from build123d import *

# Parameters (mm, degrees)
SKETCH_1_W             = 500
SKETCH_1_H             = 300
EXTRUDE_1_DEPTH        = 45
SKETCH_2_R             = 22.5
CUT_EXTRUDE_1_DEPTH    = 8
CHAMFER_1_SIZE         = 3
SKETCH_16_R            = 15.5
CUT_EXTRUDE_3_DEPTH    = 296
SKETCH_17_R            = 31
CUT_EXTRUDE_4_DEPTH    = 296
HOLE_WIZARD_M4_1_D     = 3.3
HOLE_WIZARD_M4_1_DEPTH = 11
HOLE_WIZARD_M4_1_TIP   = 0.991420021
HOLE_WIZARD_M5_1_D     = 4.2
HOLE_WIZARD_M5_1_DEPTH = 13
HOLE_WIZARD_M5_1_TIP   = 1.2618073
HOLE_WIZARD_M30_1_D    = 26.5


with BuildPart() as part:
    # 草图1 → 凸台-拉伸1 (new body)
    with BuildSketch(Plane(origin=(0, 0, 0), x_dir=(1, 0, 0), z_dir=(0, 1, 0))):
        Rectangle(SKETCH_1_W, SKETCH_1_H)
    extrude(amount=EXTRUDE_1_DEPTH)

    # 草图2 → 切除-拉伸1 (cut)
    with BuildSketch(Plane.XZ):
        with Locations(Location((190, 90, 0), (0, 0, 270))):
            Circle(SKETCH_2_R)
        with Locations(Location((-190, 90, 0), (0, 0, 90))):
            Circle(SKETCH_2_R)
        with Locations(Location((190, -90, 0), (0, 0, 270))):
            Circle(SKETCH_2_R)
        with Locations(Location((-190, -90, 0), (0, 0, 90))):
            Circle(SKETCH_2_R)
    extrude(amount=-CUT_EXTRUDE_1_DEPTH, mode=Mode.SUBTRACT)

    # 倒角1
    chamfer_1_edges = [part.edges().sort_by_distance(p)[0] for p in [
        (250, 22.5, 150),
        (-250, 22.5, 150),
        (-250, 22.5, -150),
        (250, 22.5, -150),
    ]]
    chamfer(chamfer_1_edges, length=CHAMFER_1_SIZE)

    # 草图16 → 切除-拉伸3 (cut, through all)
    with BuildSketch(Plane(origin=(0, 45, 0), x_dir=(1, 0, 0), z_dir=(0, 1, 0))):
        with Locations(Location((190, -90, 0), (0, 0, 270))):
            Circle(SKETCH_16_R)
        with Locations(Location((190, 90, 0), (0, 0, 270))):
            Circle(SKETCH_16_R)
        with Locations(Location((-190, 90, 0), (0, 0, 270))):
            Circle(SKETCH_16_R)
        with Locations(Location((-190, -90, 0), (0, 0, 270))):
            Circle(SKETCH_16_R)
    extrude(amount=-CUT_EXTRUDE_3_DEPTH, mode=Mode.SUBTRACT)

    # 草图17 → 切除-拉伸4 (cut, through all)
    with BuildSketch(Plane.XZ):
        with Locations(Location((0, 0, 0), (0, 0, 270))):
            Circle(SKETCH_17_R)
    extrude(amount=-CUT_EXTRUDE_4_DEPTH, mode=Mode.SUBTRACT)

    # M4 螺纹孔1
    with Locations(Plane(origin=(0, 45, 0), x_dir=(1, 0, 0), z_dir=(0, 1, 0))):
        with Locations((-188, 30.5), (-245, 9.5), (-188, 9.5), (-245, 30.5)):
            Hole(HOLE_WIZARD_M4_1_D / 2, depth=HOLE_WIZARD_M4_1_DEPTH)
            with Locations((0, 0, -(HOLE_WIZARD_M4_1_DEPTH + HOLE_WIZARD_M4_1_TIP / 2))):  # 118° drill point
                Cone(0, HOLE_WIZARD_M4_1_D / 2, HOLE_WIZARD_M4_1_TIP, mode=Mode.SUBTRACT)

    # M5 螺纹孔1
    with Locations(Plane(origin=(250, 0, 0), x_dir=(0, 0, -1), z_dir=(1, 0, 0))):
        with Locations((-17, 30), (17, 30)):
            Hole(HOLE_WIZARD_M5_1_D / 2, depth=HOLE_WIZARD_M5_1_DEPTH)
            with Locations((0, 0, -(HOLE_WIZARD_M5_1_DEPTH + HOLE_WIZARD_M5_1_TIP / 2))):  # 118° drill point
                Cone(0, HOLE_WIZARD_M5_1_D / 2, HOLE_WIZARD_M5_1_TIP, mode=Mode.SUBTRACT)

    # M30 螺纹孔1 (through all)
    with Locations(Plane(origin=(0, 45, 0), x_dir=(1, 0, 0), z_dir=(0, 1, 0))):
        with Locations((-127.5, 70), (-127.5, -70), (127.5, 70), (127.5, -70)):
            Hole(HOLE_WIZARD_M30_1_D / 2)


solid = part.part
Read the model definition and answer for the solid it produces. Units are mm, in the model's axes. A direction names the side the tool comes from. Round coordinates to 2 decimals unless told otherwise and drop trailing zeros. Write each loop counter-clockwise with the first axis right and the second up, starting at its lowest first coordinate (ties: lowest second). Pieces come first, ordered by that corner, then holes.
1. Determine the mould class of faces 1 (the face through (-3, 22, 150)), 2 (the face through (-250, 22, 2)), 3 (the face through (30.736, 22.185, 4.036)) for opening direction X: pulls with the +X half, pulls with the -X half, needs draft (parallel to the pull), parting line crosses it, or undercut.
2. Given pin 1 Ø2.5 at (x, z) = (-245, -30.5) entering from +Y; pin 2 Ø22.5 at (x, z) = (-199.5, 90) entering from -Y, each flat-ended and moving along its own axis, determine where each tip first touches the part or whether it passes through.
3. The part is cut by section A-A, the plane z = 90. Determine the outline of the cut face in (x, y).
4. The part is cut by section D-D, the plane x = 127.5. Determine the outline of the cut face in (y, z), then the cut area to 3 significant figures.
5. Which of the six approach directions +Z, -Z, +X, -X, +Y, -Y give full straight-line access (tool end or side, diameter ignored) to faces 4 (the face through (-3.5, 45, 31.2)), 5 (the face through (-205.21, 3.94, -106.58))?
6. Straight lines are drawn through the part: L1, parallel to Z at x = -245, y = 37.5; L2, parallel to X at y = 5.5, z = -90; L3, parallel to Z at x = -190, y = 4. For each, find the intervals that lie inside material, in ascending order.
7. The part is cut by section B-B, the plane x = 0. Determine the outline of the cut face in (y, z), then the cut area to 3 significant figures.
8. The part is cut by section C-C, the plane z = 0. Determine the outline of the cut face in (x, y).
Values:
1. face 1: needs draft
1. face 2: pulls with the -X half
1. face 3: undercut
2. pin 1: stops at y = 33.76
2. pin 2: stops at y = 8
3. outline: (-250, 0) - (-212.5, 0) - (-212.5, 8) - (-205.5, 8) - (-205.5, 45) - (-250, 45) - close; (-174.5, 8) - (-167.5, 8) - (-167.5, 0) - (167.5, 0) - (167.5, 8) - (174.5, 8) - (174.5, 45) - (-174.5, 45) - close; (205.5, 8) - (212.5, 8) - (212.5, 0) - (250, 0) - (250, 45) - (205.5, 45) - close
4. outline: (0, -150) - (45, -150) - (45, -83.25) - (0, -83.25) - close; (0, -56.75) - (45, -56.75) - (45, 56.75) - (0, 56.75) - close; (0, 83.25) - (45, 83.25) - (45, 150) - (0, 150) - close
4. area: 11,100 mm2
5. face 4: +Z, -Z, +X, -X, +Y
5. face 5: -Y
6. L1: z = -150 to -32.15, -28.85 to -11.15, -7.85 to 150
6. L2: x = -250 to -212.5, -167.5 to 167.5, 212.5 to 250
6. L3: z = -150 to -112.5, -67.5 to 67.5, 112.5 to 150
7. outline: (0, -150) - (45, -150) - (45, -31) - (0, -31) - close; (0, 31) - (45, 31) - (45, 150) - (0, 150) - close
7. area: 10,700 mm2
8. outline: (-250, 0) - (-31, 0) - (-31, 45) - (-250, 45) - close; (31, 0) - (250, 0) - (250, 45) - (31, 45) - close
